Could you check a few things on this model? Use its own coordinates, in mm. Face numbers are marked on the shaded views. Give positions to 0.01 mm unless a question says otherwise; leave off trailing zeros. Write each loop counter-clockwise with the first axis right and the second up, starting at its lowest first coordinate (ties: lowest second). Pieces come first, ordered by that corner, then holes. Notation, with made-up numbers: (69, -29) - (84, -29) arc R18 cw to (84, -12) - close; hole circle Ø6 at (-2.75, 80.5). An arc over 180 degrees is marked (long way). Answer in a Markdown table with one row per item.
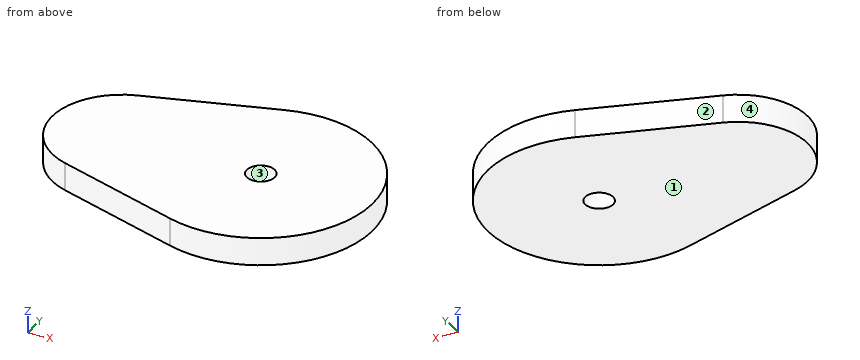
from build123d import *

# Parameters (mm, degrees)
SKETCH1_R           = 5
BOSS_EXTRUDE1_DEPTH = 10


with BuildPart() as part:
    # Sketch1 → Boss-Extrude1 (new body)
    with BuildSketch(Plane.XY):
        with BuildLine():
            Line((-57.5, 23.848480035), (-12, 38.157568057))
            ThreePointArc((-12, 38.157568057), (40, 0), (-12, -38.157568057))
            Line((-12, -38.157568057), (-57.5, -23.848480035))
            ThreePointArc((-57.5, -23.848480035), (-75, 0), (-57.5, 23.848480035))
        make_face()
        Circle(SKETCH1_R, mode=Mode.SUBTRACT)
    extrude(amount=BOSS_EXTRUDE1_DEPTH)


solid = part.part
1) We'd pull the mould along Y, two halves only. Please class the marked faces 1, 2, 3 and 4: +Y half, -Y half, draft (parallel to the pull), parting line (faces both ways), or undercut.
Check values:
| item | result |
|---|---|
| face 1 | draft |
| face 2 | +Y half |
| face 3 | undercut |
| face 4 | parting line |
2) Imagine slicing it at A-A (x = 0). List the corners of the cut face in (y, z) for me.
Check values:
| item | result |
|---|---|
| outline | (-40, 0) - (-5, 0) - (-5, 10) - (-40, 10) - close; (5, 0) - (40, 0) - (40, 10) - (5, 10) - close |
3) Imagine slicing it at C-C (z = 7.75). List the corners of the cut face in (x, y) for me.
Check values:
| item | result |
|---|---|
| outline | (-57.5, -23.85) - (-12, -38.16) arc R40 ccw (long way) to (-12, 38.16) - (-57.5, 23.85) arc R25 ccw to start; hole circle Ø10 at (0, 0) |
4) If I drill on line 1 (Y direction, x = 0, z = 4.25); line 2 (X direction, y = -0.5, z = 1.75) (3 decimals); line 3 (X direction, y = -4, z = 7.25), over which ranges is the centre line in solid material (lowest first)?
Check values:
| item | result |
|---|---|
| line 1 | y = -40 to -5, 5 to 40 |
| line 2 | x = -74.995 to -4.975, 4.975 to 39.997 |
| line 3 | x = -74.68 to -3, 3 to 39.8 |
5) Imagine slicing it at D-D (y = 9). List the corners of the cut face in (x, z) for me, then the cut area to 3 significant figures.
Check values:
| item | result |
|---|---|
| outline | (-73.32, 0) - (38.97, 0) - (38.97, 10) - (-73.32, 10) - close |
| area | 1,120 mm2 |
6) Will these pins go through, and if not, where does the flat tip stop? P1, Ø2, axis at y = -5.5, z = 3, coming from the -X side; P2, Ø6, axis at y = -4.5, z = 4.5, coming from the +X side; P3, Ø6, axis at x = -18, z = 2, coming from the +Y side.
Check values:
| item | result |
|---|---|
| P1 | stops at x = -74.59 |
| P2 | stops at x = 39.97 |
| P3 | stops at y = 37.21 |
7) Imagine slicing it at B-B (y = 0). List the corners of the cut face in (x, z) for me, then the cut area to 3 significant figures.
Check values:
| item | result |
|---|---|
| outline | (-75, 0) - (-5, 0) - (-5, 10) - (-75, 10) - close; (5, 0) - (40, 0) - (40, 10) - (5, 10) - close |
| area | 1,050 mm2 |
